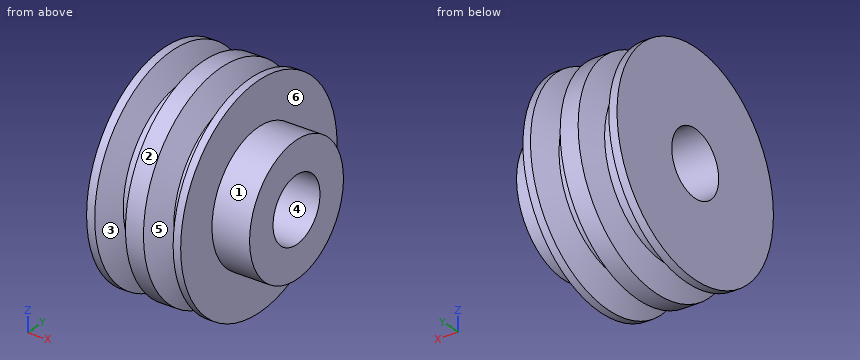
```python
from build123d import *


with BuildPart() as part:
    # Sketch1 → Revolve1 (revolve)
    with BuildSketch(Plane(origin=(0, 0, 0), x_dir=(1, 0, 0), z_dir=(0, 1, 0)), mode=Mode.PRIVATE) as revolve1_sk:
        Polygon((0, 12), (0, 40), (3.025923231, 40), (6.441608618, 30.091710395), (11.827881728, 30.091710395), (14.455332026, 40), (21.155330284, 40), (25.227878246, 30.091710395), (28.774936147, 30.091710395), (32.190621534, 40), (35, 40), (35, 24), (48.996539792, 24), (48.996539792, 12), align=None)
    revolve(revolve1_sk.sketch.rotate(Axis((0, 0, 0), (1, 0, 0)), 180), axis=Axis((0, 0, 0), (1, 0, 0)))


solid = part.part
```
Geometry check sheet. Reference: the model listing, model coordinates, mm. Face numbers are marked on the shaded views. A direction names the side the tool comes from. Give positions to 0.01 mm unless a question says otherwise; leave off trailing zeros. Write each loop counter-clockwise with the first axis right and the second up, starting at its lowest first coordinate (ties: lowest second). Pieces come first, ordered by that corner, then holes. Notation, with made-up numbers: (-7, 65.5) - (29, 65.5) arc R25 cw to (29, 102.5) - close; hole circle Ø4 at (58, 81.25). An arc over 180 degrees is marked (long way). Use a Markdown table: item, result.
Q1. Section check A-A, the plane y = 0. Enter the section's corners in (x, z).
Computed:
| item | result |
|---|---|
| outline | (0, -40) - (3.03, -40) - (6.44, -30.09) - (11.83, -30.09) - (14.46, -40) - (21.16, -40) - (25.23, -30.09) - (28.77, -30.09) - (32.19, -40) - (35, -40) - (35, -24) - (49, -24) - (49, -12) - (0, -12) - close; (0, 12) - (49, 12) - (49, 24) - (35, 24) - (35, 40) - (32.19, 40) - (28.77, 30.09) - (25.23, 30.09) - (21.16, 40) - (14.46, 40) - (11.83, 30.09) - (6.44, 30.09) - (3.03, 40) - (0, 40) - close |
Q2. Set-up check for the marked faces 1, 2 and 3: record each of +Z, -Z, +X, -X, +Y, -Y from which the full face is reachable in a straight line by a thin tool's end or side.
Computed:
| item | result |
|---|---|
| face 1 | +X |
| face 2 | +X, -X |
| face 3 | none |
Q3. Go/stop test with flat-tipped pins: P1, Ø5, axis at x = 33.5, z = 13, coming from the +Y side; P2, Ø5, axis at x = 22.5, z = -16, coming from the -Y side; P3, Ø2, axis at y = 21.5, z = -28.5, coming from the -X side; P4, Ø8, axis at x = 39.5, y = 25.5, coming from the -Z side. Record where each tip stops, or that it passes through.
Computed:
| item | result |
|---|---|
| P1 | stops at y = 38.6 |
| P2 | stops at y = -37.51 |
| P3 | stops at x = 0 |
| P4 | stops at z = -10.67 |
Q4. Thickness scan on L1, parallel to X at y = -19, z = 31; L2, parallel to Y at x = 19, z = 0; L3, parallel to X at y = -25, z = -22. Record the ranges inside material, lowest first. Write a range as [from, to].
Computed:
| item | result |
|---|---|
| L1 | x = [0, 4.28], [13.49, 22.65], [30.94, 35] |
| L2 | y = [-40, -12], [12, 40] |
| L3 | x = [0, 5.34], [12.68, 23.91], [29.88, 35] |
Q5. Section check D-D, the plane x = 23. Enter the section's corners in (y, z).
Computed:
| item | result |
|---|---|
| outline | circle Ø71.02 at (0, 0); hole circle Ø24 at (0, 0) |
Q6. Draft check along Y on the marked faces 4, 5 and 6. Enter one of: pulls with the +Y half, pulls with the -Y half, needs draft (parallel to the pull), parting line crosses it, or undercut.
Computed:
| item | result |
|---|---|
| face 4 | undercut |
| face 5 | parting line crosses it |
| face 6 | needs draft |
Q7. Section check C-C, the plane x = 9. Enter the section's corners in (y, z), then the cut area to 3 significant figures.
Computed:
| item | result |
|---|---|
| outline | circle Ø60.18 at (0, 0); hole circle Ø24 at (0, 0) |
| area | 2,390 mm² |
